The listing builds one solid part. Answer for the finished solid, in the listing's coordinates (mm). A direction names the side the tool comes from. Round coordinates to 2 decimals unless told otherwise and drop trailing zeros. Order: outer loops, then holes, each group sorted by start corner. A loop starts at its lowest first (then second) coordinate and runs counter-clockwise, first axis right, second up. Notation, with made-up numbers: (1, 43) -> (22, 43) arc R21 cw to (22, 57) -> close; hole circle Ø1 at (-35, -32). An arc over 180 degrees is marked (long way). Return JSON: item names as keys, results as strings. Group by question number.
(1) The part is cut by section D-D (x = 114). Determine the outline of the cut face in (y, z).
(2) The part is cut by section C-C (z = 13). Determine the outline of the cut face in (x, y), plus the area to 3 significant figures.
(3) The part is cut by section B-B (y = -7.5). Determine the outline of the cut face in (x, z), plus the area to 3 significant figures.
(4) Each of these flat-tipped pins is pushed along its axis until it touches: pin 1 (1.5 mm diameter, centred on x = -1, y = 21, fed in from +Z); pin 2 (1 mm diameter, centred on x = -8, y = 10, fed in from +Z); pin 3 (25 mm diameter, centred on y = -9.5, z = -9, fed in from +X); pin 4 (1.5 mm diameter, centred on x = 30.5, z = 20.5, fed in from +Y). Where does it stop, or does it pass through?
(5) Consider line 1 (Y direction, x = -29, z = 0); line 2 (X direction, y = 35.5, z = -4); line 3 (X direction, y = -16.5, z = 4.5). Determine where each line is inside the solid, lowest interval first. Write a range as [from, to].
(6) Which of the six approach directions +Z, -Z, +X, -X, +Y, -Y give full straight-line access (tool end or side, diameter ignored) to faces 1 (the face through (50.14, -0.88, -19.98)), 2 (the face through (140, 0, 0)), 3 (the face through (0, 0, 0))?
(7) The part is cut by section A-A (x = 95). Determine the outline of the cut face in (y, z).
(8) Determine the mould class of faces 4 (the face through (120, 2, 2)), 5 (the face through (-19.72, -19.524, -4.336)), 6 (the face through (90, 0, -10)) for opening direction Z: +Z half, -Z half, draft (parallel to the pull), parting line (faces both ways), or undercut.
from build123d import *

# Parameters (mm, degrees)
END_START             = -40
END_CUT_SKETCH_40_R   = 20
END_CUT_40_X_40_DEPTH = 40


with BuildPart() as part:
    # Shaft Profile Sketch → Stepped Shaft Revolve (revolve)
    with BuildSketch(Plane.XY, mode=Mode.PRIVATE) as stepped_shaft_revolve_sk:
        Polygon((-40, 0), (-40, 25), (0, 25), (0, 40), (20, 40), (20, 25), (40, 25), (40, 20), (60, 20), (60, 15), (80, 15), (80, 10), (100, 10), (100, 5), (120, 5), (120, 2.5), (140, 2.5), (140, 0), align=None)
    revolve(stepped_shaft_revolve_sk.sketch.rotate(Axis((-63.850651288, 0, 0), (1, 0, 0)), 90), axis=Axis((-63.850651288, 0, 0), (1, 0, 0)))

    # End Cut Sketch Ø40 → End Cut Ø40 x 40 (cut)
    with BuildSketch(Plane.ZY.offset(40).offset(END_START)):
        Circle(END_CUT_SKETCH_40_R)
    extrude(amount=END_CUT_40_X_40_DEPTH, mode=Mode.SUBTRACT)


solid = part.part
Answer below:
{
 "1": {"outline": "circle Ø10 at (0, 0)"},
 "2": {"outline": "(-40, -21.35) -> (0, -21.35) -> (0, -37.83) -> (20, -37.83) -> (20, -21.35) -> (40, -21.35) -> (40, -15.2) -> (60, -15.2) -> (60, -7.48) -> (80, -7.48) -> (80, 7.48) -> (60, 7.48) -> (60, 15.2) -> (40, 15.2) -> (40, 21.35) -> (20, 21.35) -> (20, 37.83) -> (0, 37.83) -> (0, 21.35) -> (-40, 21.35) -> (-40, 15.2) -> (0, 15.2) -> (0, -15.2) -> (-40, -15.2) -> close", "area": "3,770 mm²"},
 "3": {"outline": "(-40, -23.85) -> (0, -23.85) -> (0, -39.29) -> (20, -39.29) -> (20, -23.85) -> (40, -23.85) -> (40, -18.54) -> (60, -18.54) -> (60, -12.99) -> (80, -12.99) -> (80, -6.61) -> (100, -6.61) -> (100, 6.61) -> (80, 6.61) -> (80, 12.99) -> (60, 12.99) -> (60, 18.54) -> (40, 18.54) -> (40, 23.85) -> (20, 23.85) -> (20, 39.29) -> (0, 39.29) -> (0, 23.85) -> (-40, 23.85) -> (-40, 18.54) -> (0, 18.54) -> (0, -18.54) -> (-40, -18.54) -> close", "area": "4,480 mm²"},
 "4": {"pin 1": "stops at z = 14.66", "pin 2": "stops at z = 23.12", "pin 3": "stops at x = 140", "pin 4": "stops at y = 15.33"},
 "5": {"line 1": "y = [-25, -20], [20, 25]", "line 2": "x = [0, 20]", "line 3": "x = [0, 60]"},
 "6": {"face 1": "+X", "face 2": "+Z, -Z, +X, +Y, -Y", "face 3": "-X"},
 "7": {"outline": "circle Ø20 at (0, 0)"},
 "8": {"face 4": "draft", "face 5": "undercut", "face 6": "parting line"}
}
